```python
from build123d import *

# Parameters (mm, degrees)
SKETCH_2_R             = 35
EXTRUDE_1_DEPTH        = 122
SKETCH_3_R             = 7
CUT_EXTRUDE_1_DEPTH    = 132.658649545
SKETCH_4_R             = 17.5
CUT_EXTRUDE_2_DEPTH    = 116
SKETCH_5_OUTSIDE_W     = 103.422
SKETCH_5_OUTSIDE_H     = 103.422
SKETCH_5_OUTSIDE_R     = 25
CUT_EXTRUDE_3_DEPTH    = 30
SKETCH_6_OUTSIDE_W     = 103.422
SKETCH_6_OUTSIDE_H     = 103.422
SKETCH_6_OUTSIDE_R     = 25
CUT_EXTRUDE_4_DEPTH    = 84
SKETCH_7_R             = 2.1
CUT_EXTRUDE_5_DEPTH    = 105.470091414
SKETCH_8_R             = 4
CUT_EXTRUDE_6_DEPTH    = 4.2
HOLE_WIZARD_M4_1_D     = 3.3
HOLE_WIZARD_M4_1_DEPTH = 10.5
HOLE_WIZARD_M4_1_TIP   = 0.991420021
SKETCH_19_W            = 12.931297241
SKETCH_19_H            = 3
CUT_EXTRUDE_7_DEPTH    = 15
SKETCH_20_W            = 3
SKETCH_20_H            = 28.427665472
CUT_EXTRUDE_8_DEPTH    = 141.388745988
SKETCH_21_R            = 4
CUT_EXTRUDE_9_DEPTH    = 18
SKETCH_22_R            = 2.25
CUT_EXTRUDE_10_DEPTH   = 22
HOLE_WIZARD_M4_3_D     = 3.3


with BuildPart() as part:
    # 草图2 → 凸台-拉伸1 (new body)
    with BuildSketch(Plane.XY):
        with Locations(Location((0, 0, 0), (0, 0, 180))):
            Circle(SKETCH_2_R)
    extrude(amount=EXTRUDE_1_DEPTH)

    # 草图3 → 切除-拉伸1 (cut, through all)
    with BuildSketch(Plane.XY.offset(122)):
        Circle(SKETCH_3_R)
    extrude(amount=-CUT_EXTRUDE_1_DEPTH, mode=Mode.SUBTRACT)

    # 草图4 → 切除-拉伸2 (cut)
    with BuildSketch(Plane(origin=(0, 0, 0), x_dir=(-1, 0, 0), z_dir=(0, 0, -1))):
        Circle(SKETCH_4_R)
    extrude(amount=-CUT_EXTRUDE_2_DEPTH, mode=Mode.SUBTRACT)

    # 草图5 outside → 切除-拉伸3 (cut)
    with BuildSketch(Plane.XY.offset(122)):
        Rectangle(SKETCH_5_OUTSIDE_W, SKETCH_5_OUTSIDE_H)
        Circle(SKETCH_5_OUTSIDE_R, mode=Mode.SUBTRACT)
    extrude(amount=-CUT_EXTRUDE_3_DEPTH, mode=Mode.SUBTRACT)

    # 草图6 outside → 切除-拉伸4 (cut)
    with BuildSketch(Plane(origin=(0, 0, 0), x_dir=(-1, 0, 0), z_dir=(0, 0, -1))):
        Rectangle(SKETCH_6_OUTSIDE_W, SKETCH_6_OUTSIDE_H)
        with Locations(Location((0, 0, 0), (0, 0, 180))):
            Circle(SKETCH_6_OUTSIDE_R, mode=Mode.SUBTRACT)
    extrude(amount=-CUT_EXTRUDE_4_DEPTH, mode=Mode.SUBTRACT)

    # 草图7 → 切除-拉伸5 (cut, through all)
    with BuildSketch(Plane.XY.offset(92)):
        with Locations((0, 29.5)):
            Circle(SKETCH_7_R)
        with Locations((29.5, 0)):
            Circle(SKETCH_7_R)
        with Locations((0, -29.5)):
            Circle(SKETCH_7_R)
        with Locations((-29.5, 0)):
            Circle(SKETCH_7_R)
    extrude(amount=-CUT_EXTRUDE_5_DEPTH, mode=Mode.SUBTRACT)

    # 草图8 → 切除-拉伸6 (cut)
    with BuildSketch(Plane.XY.offset(92)):
        with Locations((0, 29.5)):
            Circle(SKETCH_8_R)
        with Locations((-29.5, 0)):
            Circle(SKETCH_8_R)
        with Locations((29.5, 0)):
            Circle(SKETCH_8_R)
        with Locations((0, -29.5)):
            Circle(SKETCH_8_R)
    extrude(amount=-CUT_EXTRUDE_6_DEPTH, mode=Mode.SUBTRACT)

    # M4 螺纹孔1
    with Locations(Plane(origin=(18.186533479, -10.5, 122), x_dir=(1, 0, 0), z_dir=(0, 0, 1))):
        with Locations((0, 0), (-36.373066958, 0), (-18.186533479, 31.5)):
            Hole(HOLE_WIZARD_M4_1_D / 2, depth=HOLE_WIZARD_M4_1_DEPTH)
            with Locations((0, 0, -(HOLE_WIZARD_M4_1_DEPTH + HOLE_WIZARD_M4_1_TIP / 2))):  # 118° drill point
                Cone(0, HOLE_WIZARD_M4_1_D / 2, HOLE_WIZARD_M4_1_TIP, mode=Mode.SUBTRACT)

    # 草图19 → 切除-拉伸7 (cut)
    with BuildSketch(Plane(origin=(0, 0, 0), x_dir=(-1, 0, 0), z_dir=(0, 0, -1))):
        with Locations((20.220472236, 1.5)):
            Rectangle(SKETCH_19_W, SKETCH_19_H)
    extrude(amount=-CUT_EXTRUDE_7_DEPTH, mode=Mode.SUBTRACT)

    # 草图20 → 切除-拉伸8 (cut, through all)
    with BuildSketch(Plane(origin=(-25, 0, 0), x_dir=(0, 0, -1), z_dir=(1, 0, 0))):
        with Locations((-13.5, 14.213832736)):
            Rectangle(SKETCH_20_W, SKETCH_20_H)
    extrude(amount=CUT_EXTRUDE_8_DEPTH, mode=Mode.SUBTRACT)

    # 草图21 → 切除-拉伸9 (cut)
    with BuildSketch(Plane(origin=(0, 25, 0), x_dir=(-1, 0, 0), z_dir=(0, 1, 0))):
        with Locations((21, 6)):
            Circle(SKETCH_21_R)
    extrude(amount=-CUT_EXTRUDE_9_DEPTH, mode=Mode.SUBTRACT)

    # 草图22 → 切除-拉伸10 (cut)
    with BuildSketch(Plane(origin=(0, 25, 0), x_dir=(-1, 0, 0), z_dir=(0, 1, 0))):
        with Locations(Location((21, 6, 0), (0, 0, 90))):
            Circle(SKETCH_22_R)
    extrude(amount=-CUT_EXTRUDE_10_DEPTH, mode=Mode.SUBTRACT)

    # M4 螺纹孔3 (through all)
    with Locations(Plane(origin=(-21, 0, 6), x_dir=(0, 0, 1), z_dir=(0, 1, 0))):
        with Locations((0, 0)):
            Hole(HOLE_WIZARD_M4_3_D / 2)


solid = part.part
```
CAD build for the part. Positions are in the model's coordinates, mm. A direction names the side the tool comes from. Coordinates: 2 decimals unless noted, no trailing zeros. Order: outer loops, then holes, each group sorted by start corner. A loop starts at its lowest first (then second) coordinate and runs counter-clockwise, first axis right, second up. Notation, with made-up numbers: (83.5, -37.75) - (109.5, -37.75) arc R26 ccw to (109.5, -16.75) - close; hole circle Ø9 at (52, 64.25). An arc over 180 degrees is marked (long way). Use a Markdown table: item, result. Add a question column.
(1) Drill centre lines: line 1 along Y through (x, z) = (0, 120.8); line 2 along Z through (x, y) = (17, 8); line 3 along X through (y, z) = (6, 6). Where is each one in solid material? Low to high. Write a range as [from, to].
(2) Saw through at A-A (x = -13). Give the cut face in (y, z), then the cut area to 3 significant figures.
(3) Saw through at D-D (x = 23.5). Give the cut face in (y, z).
(4) Saw through at B-B (y = -23.5). Give the cut face in (x, z), then the cut area to 3 significant figures.
(5) Which spindle directions (+Z, -Z, +X, -X, +Y, -Y) get a long thin tool onto all of the face, cutting with end or side? Do faces 4 (the face through (0, 18, 12)), 5 (the face through (-0.521, 33.466, 89.929)), 6 (the face through (-23, 11, 84)). Say none if no direction does.
(6) Pull direction X, two halves, no side cores. Call faces 1 (the face through (2, -31, 87.8)), 2 (the face through (7.587, 34.168, 87.944)), 3 (the face through (17, 5, 0)): +X half, -X half, draft (parallel to the pull), parting line (faces both ways), or undercut.
(7) Flat gauge pins, fed straight in: pin 1 (5 mm diameter, centred on x = -1.5, z = 27.5, fed in from +Y); pin 2 (8 mm diameter, centred on y = -8.5, z = 33, fed in from -X); pin 3 (2.5 mm diameter, centred on x = 0.5, y = 31, fed in from +Z); pin 4 (4.5 mm diameter, centred on x = -18.19, y = -10.5, fed in from +Z). Where does each tip first touch, or does it go through?
(8) Saw through at C-C (z = 62). Give the cut face in (x, y), then the cut area to 3 significant figures.
Solved:
| question | item | result |
|---|---|---|
| 1 | line 1 | y = [-25, -7], [7, 19.35], [22.65, 25] |
| 1 | line 2 | z = [0, 12], [15, 122] |
| 1 | line 3 | x = [-24.27, -23.25], [-18.75, -16.44], [16.44, 24.27] |
| 2 | outline | (-32.5, 84) - (-21.35, 84) - (-21.35, 0) - (-11.72, 0) - (-11.72, 116) - (11.72, 116) - (11.72, 15) - (21.35, 15) - (21.35, 84) - (32.5, 84) - (32.5, 92) - (21.35, 92) - (21.35, 122) - (-21.35, 122) - (-21.35, 92) - (-32.5, 92) - close; (11.72, 0) - (21.35, 0) - (21.35, 12) - (11.72, 12) - close |
| 2 | area | 2,640 mm² |
| 3 | outline | (-25.94, 84) - (-8.53, 84) - (-8.53, 0) - (8.53, 0) - (8.53, 12) - (0, 12) - (0, 15) - (8.53, 15) - (8.53, 84) - (25.94, 84) - (25.94, 92) - (8.53, 92) - (8.53, 122) - (-8.53, 122) - (-8.53, 92) - (-25.94, 92) - close |
| 4 | outline | (-25.94, 84) - (-8.53, 84) - (-8.53, 0) - (8.53, 0) - (8.53, 84) - (25.94, 84) - (25.94, 92) - (8.53, 92) - (8.53, 122) - (-8.53, 122) - (-8.53, 92) - (-25.94, 92) - close |
| 4 | area | 2,360 mm² |
| 5 | face 4 | +X, -X, +Y |
| 5 | face 5 | +Z |
| 5 | face 6 | -Z |
| 6 | face 1 | undercut |
| 6 | face 2 | parting line |
| 6 | face 3 | draft |
| 7 | pin 1 | stops at y = 25 |
| 7 | pin 2 | stops at x = -24.59 |
| 7 | pin 3 | stops at z = 87.8 |
| 7 | pin 4 | stops at z = 122 |
| 8 | outline | circle Ø50 at (0, 0); hole circle Ø35 at (0, 0) |
| 8 | area | 1,000 mm² |
